from build123d import *

# Parameters (mm, degrees)
SKETCH2_R                   = 17
CUT_EXTRUDE1_DEPTH          = 2
CUT_EXTRUDE2_DEPTH          = 4.5
CUT_EXTRUDE3_DEPTH          = 3.5
SKETCH5_R                   = 3
CUT_EXTRUDE4_DEPTH          = 11
SKETCH7_R                   = 4.5
CUT_EXTRUDE5_DEPTH          = 6
SKETCH8_R                   = 3.5
CUT_EXTRUDE6_DEPTH          = 2.5
SKETCH9_R                   = 2.6
CUT_EXTRUDE7_DEPTH          = 46.617978912
CHAMFER1_SIZE               = 1
SKETCH10_R                  = 14.5
SKETCH10_R_2                = 6.5
CUT_EXTRUDE8_DEPTH          = 0.5
M8_TAPPED_HOLE1_D           = 6.8
M8_TAPPED_HOLE1_DEPTH       = 10
M8_TAPPED_HOLE1_CSINK_D     = 8.05
M8_TAPPED_HOLE1_CSINK_ANGLE = 90
M8_TAPPED_HOLE1_TIP         = 2.042926105


with BuildPart() as part:
    # Sketch1 → Revolve1 (revolve)
    with BuildSketch(Plane.XY, mode=Mode.PRIVATE) as revolve1_sk:
        Polygon((0, 9.6), (0, 0), (3.5, -8.4), (20, -8.4), (20, 9.6), align=None)
    revolve(revolve1_sk.sketch.rotate(Axis((20, -8.4, 0), (0, 1, 0)), 180), axis=Axis((20, -8.4, 0), (0, 1, 0)))

    # Sketch2 → Cut-Extrude1 (cut)
    with BuildSketch(Plane(origin=(0, 9.6, 0), x_dir=(1, 0, 0), z_dir=(0, 1, 0))):
        with Locations(Location((20, 0, 0), (0, 0, 180))):
            Circle(SKETCH2_R)
    extrude(amount=-CUT_EXTRUDE1_DEPTH, mode=Mode.SUBTRACT)

    # Sketch3 → Cut-Extrude2 (cut)
    with BuildSketch(Plane(origin=(0, 7.6, 0), x_dir=(1, 0, 0), z_dir=(0, 1, 0))):
        with BuildLine():
            Line((24, 4.5), (24, -4.5))
            ThreePointArc((24, -4.5), (20, -8.5), (16, -4.5))
            Line((16, -4.5), (16, 4.5))
            ThreePointArc((16, 4.5), (20, 8.5), (24, 4.5))
        make_face()
    extrude(amount=-CUT_EXTRUDE2_DEPTH, mode=Mode.SUBTRACT)

    # Sketch4 → Cut-Extrude3 (cut)
    with BuildSketch(Plane(origin=(0, 7.6, 0), x_dir=(1, 0, 0), z_dir=(0, 1, 0))):
        with BuildLine():
            ThreePointArc((31.66726189, 11.66726189), (20, 16.5), (8.33273811, 11.66726189))
            ThreePointArc((8.33273811, 11.66726189), (8.33273811, 8.131727984), (11.868272016, 8.131727984))
            ThreePointArc((11.868272016, 8.131727984), (20, 11.5), (28.131727984, 8.131727984))
            ThreePointArc((28.131727984, 8.131727984), (31.66726189, 8.131727984), (31.66726189, 11.66726189))
        make_face()
    extrude(amount=-CUT_EXTRUDE3_DEPTH, mode=Mode.SUBTRACT)

    # Sketch5 → Cut-Extrude4 (cut)
    with BuildSketch(Plane(origin=(0, 7.6, 0), x_dir=(1, 0, 0), z_dir=(0, 1, 0))):
        with Locations(Location((6, 0, 0), (0, 0, 180))):
            Circle(SKETCH5_R)
        with Locations((34, 0)):
            Circle(SKETCH5_R)
    extrude(amount=-CUT_EXTRUDE4_DEPTH, mode=Mode.SUBTRACT)

    # Sketch7 → Cut-Extrude5 (cut)
    with BuildSketch(Plane.XZ.offset(8.4)):
        with Locations((20, 0)):
            Circle(SKETCH7_R)
    extrude(amount=-CUT_EXTRUDE5_DEPTH, mode=Mode.SUBTRACT)

    # Sketch8 → Cut-Extrude6 (cut)
    with BuildSketch(Plane(origin=(0, 3.1, 0), x_dir=(1, 0, 0), z_dir=(0, 1, 0))):
        with Locations(Location((20, 0, 0), (0, 0, 180))):
            Circle(SKETCH8_R)
    extrude(amount=-CUT_EXTRUDE6_DEPTH, mode=Mode.SUBTRACT)

    # Sketch9 → Cut-Extrude7 (cut, through all)
    with BuildSketch(Plane(origin=(0, 0.6, 0), x_dir=(1, 0, 0), z_dir=(0, 1, 0))):
        with Locations(Location((20, 0, 0), (0, 0, 180))):
            Circle(SKETCH9_R)
    extrude(amount=-CUT_EXTRUDE7_DEPTH, mode=Mode.SUBTRACT)

    # Chamfer1
    chamfer1_edges = [part.edges().sort_by_distance(p)[0] for p in [
        (22.6, -2.4, 0),
    ]]
    chamfer(chamfer1_edges, length=CHAMFER1_SIZE)

    # Sketch10 → Cut-Extrude8 (cut)
    with BuildSketch(Plane.XZ.offset(8.4)):
        with Locations((20, 0)):
            Circle(SKETCH10_R)
        with Locations((20, 0)):
            Circle(SKETCH10_R_2, mode=Mode.SUBTRACT)
    extrude(amount=-CUT_EXTRUDE8_DEPTH, mode=Mode.SUBTRACT)

    # M8 Tapped Hole1
    with Locations(Plane(origin=(0, -7.100591716, 17.041420118), x_dir=(1, 0, 0), z_dir=(0, -0.38461538461538547, 0.9230769230769227))):
        with Locations((20, 3.142307692)):
            CounterSinkHole(M8_TAPPED_HOLE1_D / 2, M8_TAPPED_HOLE1_CSINK_D / 2, depth=M8_TAPPED_HOLE1_DEPTH, counter_sink_angle=M8_TAPPED_HOLE1_CSINK_ANGLE)
            with Locations((0, 0, -(M8_TAPPED_HOLE1_DEPTH + M8_TAPPED_HOLE1_TIP / 2))):  # 118° drill point
                Cone(0, M8_TAPPED_HOLE1_D / 2, M8_TAPPED_HOLE1_TIP, mode=Mode.SUBTRACT)


solid = part.part
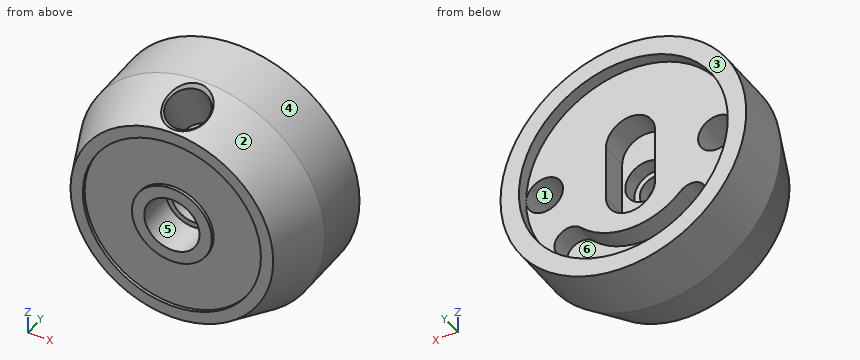
The model under review builds one solid part; all positions refer to its coordinate system, in mm. Face numbers are marked on the shaded views. A direction names the side the tool comes from. Give positions to 0.01 mm unless a question says otherwise; leave off trailing zeros. Write each loop counter-clockwise with the first axis right and the second up, starting at its lowest first coordinate (ties: lowest second). Pieces come first, ordered by that corner, then holes. Notation, with made-up numbers: M -0.75,-15 L 38.25,-15 A23 cw 38.25,-2 Z; hole C 76,75.5 d2. An arc over 180 degrees is marked long. One line per question, with ' | ' between items. Start each with the question number.
Item 1: For the marked faces 4, 5 and 6, list the 3-axis set-ups (+Z, -Z, +X, -X, +Y, -Y) from which the entire face can be reached by the end or side of a thin tool; tool diameter is ignored.
Item 2: For pin 1 (1 mm diameter, centred on x = 21, y = -6.5, fed in from +Z); pin 2 (2.5 mm diameter, centred on x = 23.5, z = -11, fed in from +Y); pin 3 (3.5 mm diameter, centred on x = 34, z = 0, fed in from +Y), all flat-tipped, find the tip position at first contact; note any pin that passes through.
Item 3: Draft analysis for pull direction Z (two halves, no side actions). For the marked faces 1, 2 and 3, state which applies: released by +Z, released by -Z, zero draft, split by the parting line, or undercut.
Item 4: We need section A-A on y = 5.25. Write out the cut boundary in (x, z).
Item 5: We need section B-B on y = 1.5. Give the number of separate pieces and of enclosed holes in the cut face, plus the area to 3 significant figures.
Item 6: Wall thickness on line 1 (Z direction, x = 20, y = -8.2); line 2 (Y direction, x = 17.5, z = -7.5); line 3 (X direction, y = -1, z = 10): over which ranges is each line inside the solid? List them lowest first. Write a range as from..to.
Results found:
1) face 4: +Y, -Y | face 5: -Y | face 6: +Y
2) pin 1: stops at z = 16.48 | pin 2: stops at y = 7.6 | pin 3: stops at y = -3.4
3) face 1: undercut | face 2: split by the parting line | face 3: zero draft
4) outline: C 20,0 d40; hole C 6,0 d6; hole M 8.33,-11.67 A16.5 ccw 31.67,-11.67 A2.5 ccw 28.13,-8.13 A11.5 cw 11.87,-8.13 A2.5 ccw Z; hole M 16,-4.5 A4 ccw 24,-4.5 L 24,4.5 A4 ccw 16,4.5 Z; hole C 34,0 d6
5) separate pieces: 1 | enclosed holes: 4 | area: 1,140 mm2
6) line 1: z = -16.58..-14.5, -6.5..-4.5, 4.5..6.5, 14.5..16.58 | line 2: y = -7.9..3.1 | line 3: x = 3.16..16.61, 23.39..36.84
